```python
from build123d import *

# Parameters (mm, degrees)
SKETCH_1_W          = 43
SKETCH_1_H          = 22
EXTRUDE_1_DEPTH     = 0.4
SKETCH_2_R          = 3
CUT_EXTRUDE_1_DEPTH = 0.4


with BuildPart() as part:
    # 草图1 → 凸台-拉伸1 (new body)
    with BuildSketch(Plane.XY):
        Rectangle(SKETCH_1_W, SKETCH_1_H)
    extrude(amount=EXTRUDE_1_DEPTH)

    # 草图2 → 切除-拉伸1 (cut)
    with BuildSketch(Plane.XY.offset(0.4)):
        Circle(SKETCH_2_R)
        with Locations((-14, 0)):
            Circle(SKETCH_2_R)
        with Locations((14, 0)):
            Circle(SKETCH_2_R)
    extrude(amount=-CUT_EXTRUDE_1_DEPTH, mode=Mode.SUBTRACT)


solid = part.part
```
Could you check a few things on this model? Use its own coordinates, in mm. Coordinates: 2 decimals unless noted, no trailing zeros. Write each loop counter-clockwise with the first axis right and the second up, starting at its lowest first coordinate (ties: lowest second). Pieces come first, ordered by that corner, then holes. Notation, with made-up numbers: (-6.75, 1) -> (41.25, 1) arc R22 cw to (41.25, 33) -> close; hole circle Ø11 at (-9, 6.5). An arc over 180 degrees is marked (long way). Return JSON: item names as keys, results as strings.
(1) Imagine slicing it at C-C, the plane z = 0.2. Please give me the cut outline in (x, y), then the cut area to 3 significant figures.
Numbers:
{"outline": "(-21.5, -11) -> (21.5, -11) -> (21.5, 11) -> (-21.5, 11) -> close; hole circle Ø6 at (-14, 0); hole circle Ø6 at (0, 0); hole circle Ø6 at (14, 0)", "area": "861 mm2"}
(2) We'd pull the mould along X, two halves only. Please class faces 1 (the flat face through (4, 0, 0.4)), 2 (the cylindrical face through (-3, 0.1, 0.2)): +X half, -X half, draft (parallel to the pull), parting line (faces both ways), or undercut.
Numbers:
{"face 1": "draft", "face 2": "undercut"}
(3) I need wall thicknesses on L1, parallel to Y at x = -14, z = 0.3; L2, parallel to X at y = -2.25, z = 0.25; L3, parallel to Y at x = 13, z = 0.25. Which ranges of each line are inside material? Lowest first, please.
Numbers:
{"L1": "y = -11 to -3, 3 to 11", "L2": "x = -21.5 to -15.98, -12.02 to -1.98, 1.98 to 12.02, 15.98 to 21.5", "L3": "y = -11 to -2.83, 2.83 to 11"}
(4) Imagine slicing it at B-B, the plane x = 14. Please give me the cut outline in (y, z).
Numbers:
{"outline": "(-11, 0) -> (-3, 0) -> (-3, 0.4) -> (-11, 0.4) -> close; (3, 0) -> (11, 0) -> (11, 0.4) -> (3, 0.4) -> close"}
(5) Imagine slicing it at A-A, the plane y = 0. Please give me the cut outline in (x, z), then the cut area to 3 significant figures.
Numbers:
{"outline": "(-21.5, 0) -> (-17, 0) -> (-17, 0.4) -> (-21.5, 0.4) -> close; (-11, 0) -> (-3, 0) -> (-3, 0.4) -> (-11, 0.4) -> close; (3, 0) -> (11, 0) -> (11, 0.4) -> (3, 0.4) -> close; (17, 0) -> (21.5, 0) -> (21.5, 0.4) -> (17, 0.4) -> close", "area": "10.0 mm2"}
